from build123d import *

# Parameters (mm, degrees)
GB_6728_1986_070_X_50_X_3_1_DEPTH = 1139.5
CUT_EXTRUDE_1_DEPTH               = 575.578160479
CUT_EXTRUDE_1_DEPTH_BACK          = 575.578160479
SKETCH_5_W                        = 71
SKETCH_5_H                        = 60
CUT_EXTRUDE_4_DEPTH               = 575.578160479


with BuildPart() as part:
    # Sketch1 → Gb／6728-1986矩形空心型钢 070 X 50 X 3(1) (new body)
    with BuildSketch(Plane.YZ.offset(-569.75)):
        with BuildLine():
            Line((-19, -35), (19, -35))
            ThreePointArc((19, -35), (23.242640687, -33.242640687), (25, -29))
            Line((25, -29), (25, 29))
            ThreePointArc((25, 29), (23.242640687, 33.242640687), (19, 35))
            Line((19, 35), (-19, 35))
            ThreePointArc((-19, 35), (-23.242640687, 33.242640687), (-25, 29))
            Line((-25, 29), (-25, -29))
            ThreePointArc((-25, -29), (-23.242640687, -33.242640687), (-19, -35))
        make_face()
        with BuildLine():
            Line((-19, -32), (19, -32))
            ThreePointArc((19, -32), (21.121320344, -31.121320344), (22, -29))
            Line((22, -29), (22, 29))
            ThreePointArc((22, 29), (21.121320344, 31.121320344), (19, 32))
            Line((19, 32), (-19, 32))
            ThreePointArc((-19, 32), (-21.121320344, 31.121320344), (-22, 29))
            Line((-22, 29), (-22, -29))
            ThreePointArc((-22, -29), (-21.121320344, -31.121320344), (-19, -32))
        make_face(mode=Mode.SUBTRACT)
    extrude(amount=GB_6728_1986_070_X_50_X_3_1_DEPTH)

    # 草图2 → 切除-拉伸1 (cut, two sides: drawn at the far end of the back side and taken through both)
    with BuildSketch(Plane(origin=(0, 0, -35), x_dir=(-1, 0, 0), z_dir=(0, 0, -1)).offset(-CUT_EXTRUDE_1_DEPTH_BACK)):
        Polygon((513.25, -25), (513.25, -19), (517.727357684, -17.498605391), (560.795284633, -12.971983864), (569.75, -3.026764911), (574.75, -3.026764911), (574.75, -30), (513.25, -30), align=None)
    extrude(amount=CUT_EXTRUDE_1_DEPTH + CUT_EXTRUDE_1_DEPTH_BACK, mode=Mode.SUBTRACT)

    # 草图5 → 切除-拉伸4 (cut, through all)
    with BuildSketch(Plane.XY.offset(35)):
        with Locations((539.25, 0)):
            Rectangle(SKETCH_5_W, SKETCH_5_H)
    extrude(amount=-CUT_EXTRUDE_4_DEPTH, mode=Mode.SUBTRACT)


solid = part.part
Design review of the part built by this model. Coordinates are the model's own, in mm. A direction names the side the tool comes from. Give positions to 0.01 mm unless a question says otherwise; leave off trailing zeros. Order: outer loops, then holes, each group sorted by start corner. A loop starts at its lowest first (then second) coordinate and runs counter-clockwise, first axis right, second up.
1. To check wall thickness, follow L1, parallel to Z at x = 240.5, y = 15.5; L2, parallel to Y at x = -138, z = -10; L3, parallel to Z at x = 423, y = 20.5. State the ranges of each line that lie inside material, in increasing order.
Solution:
L1: z = -35 to -32, 32 to 35
L2: y = -25 to -22, 22 to 25
L3: z = -34.81 to -31.6, 31.6 to 34.81
2. Tool access review of faces 1 (the flat face through (-41, 0, -35)), 2 (the flat face through (-41, 0, 32)): name each direction out of +Z, -Z, +X, -X, +Y, -Y from which nothing blocks a thin tool from reaching the whole face with its end or side.
Solution:
face 1: -Z, +X, -X, +Y, -Y
face 2: +X, -X
3. Mouldability with a two-part tool opening along Y and no side actions: class faces 3 (the flat face through (-41, 25, 0)), 4 (the flat face through (-12, -25, 0)), 5 (the flat face through (-41, 0, 35)), 6 (the flat face through (-41, 22, 0)) as +Y half, -Y half, draft (parallel to the pull), parting line (faces both ways), or undercut.
Solution:
face 3: +Y half
face 4: -Y half
face 5: draft
face 6: undercut
4. Add section C-C, the plane x = 50. State the section outline as (y, z) points.
Solution:
outline: (-25, -29) arc R6 ccw to (-19, -35) - (19, -35) arc R6 ccw to (25, -29) - (25, 29) arc R6 ccw to (19, 35) - (-19, 35) arc R6 ccw to (-25, 29) - close; hole (-22, -29) arc R3 ccw to (-19, -32) - (19, -32) arc R3 ccw to (22, -29) - (22, 29) arc R3 ccw to (19, 32) - (-19, 32) arc R3 ccw to (-22, 29) - close
5. Add section B-B, the plane y = 11. State the section outline as (x, z) points, then the cut area to 3 significant figures.
Solution:
outline: (-569.75, -35) - (503.75, -35) - (503.75, -32) - (-569.75, -32) - close; (-569.75, 32) - (503.75, 32) - (503.75, 35) - (-569.75, 35) - close
area: 6,440 mm2
6. For pin 1 Ø5 at (y, z) = (-22, -2) entering from -X, flat-tipped, find the tip position at first contact; note if it passes through.
Solution:
pin 1: stops at x = -513.25
7. Add section A-A, the plane z = -5.5. State the section outline as (x, y) points, then the cut area to 3 significant figures.
Solution:
outline: (-569.75, 22) - (503.75, 22) - (503.75, 25) - (-569.75, 25) - close; (-513.25, -25) - (503.75, -25) - (503.75, -22) - (-513.25, -22) - close
area: 6,270 mm2
